Source: CAD feature listing. Evaluate the final solid. Frame: model axes, mm. A direction names the side the tool comes from. Give positions to 0.01 mm unless a question says otherwise; leave off trailing zeros. Write each loop counter-clockwise with the first axis right and the second up, starting at its lowest first coordinate (ties: lowest second). Pieces come first, ordered by that corner, then holes. Notation, with made-up numbers: (75.25, 56) -> (87.25, 56) arc R24 ccw to (87.25, 84) -> close; hole circle Ø2 at (-33, -26.5). An arc over 180 degrees is marked (long way). Answer as a JSON object with one key per item and string values. Group by question number.
Item 1: Section query B-B on z = 3.5. Return the cut outline in (x, y), plus the area to 3 significant figures.
Item 2: Pull-direction query (Y, two-part tool) for faces 3 (the face through (9.98, 5, 4)), 4 (the face through (4, -2, 5)), 5 (the face through (6.39, 2, 5)); classes: pulls with the +Y half, pulls with the -Y half, needs draft (parallel to the pull), parting line crosses it, or undercut.
Item 3: Section query A-A on y = 3.49. Return the cut outline in (x, z).
Item 4: Ray query, probe 1 along Y at (x, z) = (5.25, 6.75); probe 2 along X at (y, z) = (6.5, 6); probe 3 along Y at (x, z) = (0.25, 5). Return the intervals inside material, ascending. Write a range as from..to.
Item 5: Access query for faces 1 (the face through (7, 4, 10)), 2 (the face through (4, 6.98, 5)). Directions: +Z, -Z, +X, -X, +Y, -Y. A direction counts if a zero-diameter tool reaches every point of the face in a straight line with its end or side. Return the directions, or none.
Item 6: Section query C-C on y = 0.5. Return the cut outline in (x, z), plus the area to 3 significant figures.
Item 7: Section query D-D on z = 5. Return the cut outline in (x, y).
from build123d import *

# Parameters (mm, degrees)
BOSS_EXTRUDE1_DEPTH = 10
SKETCH4_R           = 1.3
CUT_EXTRUDE2_DEPTH  = 19.004466113


with BuildPart() as part:
    # Sketch1 → Boss-Extrude1 (new body)
    with BuildSketch(Plane.XY):
        Polygon((-2, 8.98), (6.39, 8.98), (9.98, 8.98), (9.98, -2), (6.39, -2), (-2, -2), align=None)
        Polygon((1.59, 0), (4.8, 0), (6.39, 0), (6.39, 6.98), (4.8, 6.98), (1.59, 6.98), (1.59, 3.49), align=None, mode=Mode.SUBTRACT)
    extrude(amount=BOSS_EXTRUDE1_DEPTH)

    # Sketch4 → Cut-Extrude2 (cut, through all)
    with BuildSketch(Plane(origin=(9.98, 0, 0), x_dir=(0, 0, -1), z_dir=(1, 0, 0))):
        with Locations((-5, 3.49)):
            Circle(SKETCH4_R)
    extrude(amount=-CUT_EXTRUDE2_DEPTH, mode=Mode.SUBTRACT)


solid = part.part
Worked answers:
{
 "1": {"outline": "(-2, -2) -> (9.98, -2) -> (9.98, 8.98) -> (-2, 8.98) -> close; hole (1.59, 0) -> (6.39, 0) -> (6.39, 6.98) -> (1.59, 6.98) -> close", "area": "98.0 mm^2"},
 "2": {"face 3": "needs draft", "face 4": "pulls with the -Y half", "face 5": "undercut"},
 "3": {"outline": "(-2, 0) -> (1.59, 0) -> (1.59, 3.7) -> (-2, 3.7) -> close; (-2, 6.3) -> (1.59, 6.3) -> (1.59, 10) -> (-2, 10) -> close; (6.39, 0) -> (9.98, 0) -> (9.98, 3.7) -> (6.39, 3.7) -> close; (6.39, 6.3) -> (9.98, 6.3) -> (9.98, 10) -> (6.39, 10) -> close"},
 "4": {"probe 1": "-2..0, 6.98..8.98", "probe 2": "-2..1.59, 6.39..9.98", "probe 3": "-2..2.19, 4.79..8.98"},
 "5": {"face 1": "+Z, +X, -X, +Y, -Y", "face 2": "+Z, -Z"},
 "6": {"outline": "(-2, 0) -> (1.59, 0) -> (1.59, 10) -> (-2, 10) -> close; (6.39, 0) -> (9.98, 0) -> (9.98, 10) -> (6.39, 10) -> close", "area": "71.8 mm^2"},
 "7": {"outline": "(-2, -2) -> (9.98, -2) -> (9.98, 2.19) -> (6.39, 2.19) -> (6.39, 0) -> (1.59, 0) -> (1.59, 2.19) -> (-2, 2.19) -> close; (-2, 4.79) -> (1.59, 4.79) -> (1.59, 6.98) -> (6.39, 6.98) -> (6.39, 4.79) -> (9.98, 4.79) -> (9.98, 8.98) -> (-2, 8.98) -> close"}
}
